from build123d import *

# Parameters (mm, degrees)
SKETCH_1_W          = 101
SKETCH_1_H          = 130
EXTRUDE_1_DEPTH     = 11
CUT_EXTRUDE_1_DEPTH = 8
CUT_EXTRUDE_2_DEPTH = 8
CUT_EXTRUDE_3_REACH = 1271.625
SKETCH_4_W          = 4
SKETCH_4_H          = 32
CUT_EXTRUDE_4_REACH = 1273.161
SKETCH_5_W          = 4
SKETCH_5_H          = 32
SKETCH_6_R          = 36
EXTRUDE_2_DEPTH     = 5
SKETCH_7_R          = 14
EXTRUDE_3_DEPTH     = 4.5
SKETCH_8_R          = 32
CUT_EXTRUDE_5_DEPTH = 5
SKETCH_9_R          = 11
CUT_EXTRUDE_6_DEPTH = 5.6
SKETCH_10_R         = 9
CUT_EXTRUDE_7_DEPTH = 0.5
HOLE_WIZARD_M6_1_D  = 5
FILLET_1_R          = 5
CHAMFER_1_SIZE      = 1
FILLET_2_R          = 2
FILLET_3_R          = 4
FILLET_4_R          = 10


with BuildPart() as part:
    # 草图1 → 凸台-拉伸1 (new body)
    with BuildSketch(Plane(origin=(1263, 0, 0), x_dir=(0, 0, -1), z_dir=(1, 0, 0))):
        with Locations((11, -6.6)):
            Rectangle(SKETCH_1_W, SKETCH_1_H)
    extrude(amount=-EXTRUDE_1_DEPTH)

    # 草图2 → 切除-拉伸1 (cut)
    with BuildSketch(Plane(origin=(1263, 0, 0), x_dir=(0, 0, -1), z_dir=(1, 0, 0))):
        with BuildLine():
            Line((44.5, 25.256406461), (44.5, 42.4))
            Line((44.5, 42.4), (-14.5, 42.4))
            Line((-14.5, 42.4), (-14.5, 15.4))
            Line((-14.5, 15.4), (-34.5, 15.4))
            Line((-34.5, 15.4), (-34.5, -48.6))
            ThreePointArc((-34.5, -48.6), (-29.227922061, -61.327922061), (-16.5, -66.6))
            Line((-16.5, -66.6), (38.5, -66.6))
            ThreePointArc((38.5, -66.6), (51.227922061, -61.327922061), (56.5, -48.6))
            Line((56.5, -48.6), (56.5, 15.458447489))
            ThreePointArc((56.5, 15.458447489), (48.17544468, 17.510439768), (44.5, 25.256406461))
        make_face()
    extrude(amount=-CUT_EXTRUDE_1_DEPTH, mode=Mode.SUBTRACT)

    # 草图3 → 切除-拉伸2 (cut)
    with BuildSketch(Plane(origin=(1263, 0, 0), x_dir=(0, 0, -1), z_dir=(1, 0, 0))):
        with BuildLine():
            Line((42, 55.4), (-20, 55.4))
            ThreePointArc((-20, 55.4), (-25, 50.4), (-20, 45.4))
            Line((-20, 45.4), (42, 45.4))
            ThreePointArc((42, 45.4), (47, 50.4), (42, 55.4))
        make_face()
    extrude(amount=-CUT_EXTRUDE_2_DEPTH, mode=Mode.SUBTRACT)

    # 草图4 → 切除-拉伸3 (cut, up to next)
    with BuildSketch(Plane.XZ.offset(-42.4), mode=Mode.PRIVATE) as cut_extrude_3_sk1:
        with Locations((1261, -11)):
            Rectangle(SKETCH_4_W, SKETCH_4_H)
    cut_extrude_3_tool1 = extrude(cut_extrude_3_sk1.sketch, amount=-CUT_EXTRUDE_3_REACH, mode=Mode.PRIVATE) & part.part
    add(cut_extrude_3_tool1.solids().sort_by_distance((1261, 42.4, -11))[0], mode=Mode.SUBTRACT)

    # 草图5 → 切除-拉伸4 (cut, up to next)
    with BuildSketch(Plane(origin=(0, 58.4, 0), x_dir=(-1, 0, 0), z_dir=(0, 1, 0)), mode=Mode.PRIVATE) as cut_extrude_4_sk1:
        with Locations((-1261, -11)):
            Rectangle(SKETCH_5_W, SKETCH_5_H)
    cut_extrude_4_tool1 = extrude(cut_extrude_4_sk1.sketch, amount=-CUT_EXTRUDE_4_REACH, mode=Mode.PRIVATE) & part.part
    add(cut_extrude_4_tool1.solids().sort_by_distance((1261, 58.4, -11))[0], mode=Mode.SUBTRACT)

    # 草图6 → 凸台-拉伸2 (add)
    with BuildSketch(Plane.ZY.offset(-1252)):
        with Locations((-11, -25.6)):
            Circle(SKETCH_6_R)
    extrude(amount=EXTRUDE_2_DEPTH)

    # 草图7 → 凸台-拉伸3 (add)
    with BuildSketch(Plane.ZY.offset(-1247)):
        with Locations(Location((-11, -25.6, 0), (0, 0, 180))):
            Circle(SKETCH_7_R)
    extrude(amount=EXTRUDE_3_DEPTH)

    # 草图8 → 切除-拉伸5 (cut)
    with BuildSketch(Plane(origin=(1255, 0, 0), x_dir=(0, 0, -1), z_dir=(1, 0, 0))):
        with Locations(Location((11, -25.6, 0), (0, 0, 180))):
            Circle(SKETCH_8_R)
    extrude(amount=-CUT_EXTRUDE_5_DEPTH, mode=Mode.SUBTRACT)

    # 草图9 → 切除-拉伸6 (cut)
    with BuildSketch(Plane(origin=(1250, 0, 0), x_dir=(0, 0, -1), z_dir=(1, 0, 0))):
        with Locations(Location((11, -25.6, 0), (0, 0, 180))):
            Circle(SKETCH_9_R)
    extrude(amount=-CUT_EXTRUDE_6_DEPTH, mode=Mode.SUBTRACT)

    # 草图10 → 切除-拉伸7 (cut)
    with BuildSketch(Plane(origin=(1244.4, 0, 0), x_dir=(0, 0, -1), z_dir=(1, 0, 0))):
        with Locations(Location((11, -25.6, 0), (0, 0, 180))):
            Circle(SKETCH_10_R)
    extrude(amount=-CUT_EXTRUDE_7_DEPTH, mode=Mode.SUBTRACT)

    # M6 螺纹孔1 (through all)
    with Locations(Plane(origin=(1263, 0, 0), x_dir=(0, 0, -1), z_dir=(1, 0, 0))):
        with Locations((53.5, 41.4), (-25.5, 41.4), (-25.5, 21.4), (-33.5, -65.6), (55.5, -65.6), (53.5, 21.4)):
            Hole(HOLE_WIZARD_M6_1_D / 2)

    # 圆角1
    fillet_1_edges = [part.edges().sort_by_distance(p)[0] for p in [
        (1257.5, -71.6, 39.5),
        (1257.5, 58.4, 39.5),
        (1257.5, 58.4, -61.5),
        (1257.5, -71.6, -61.5),
    ]]
    fillet(fillet_1_edges, radius=FILLET_1_R)

    # 倒角1
    chamfer_1_edges = [part.edges().sort_by_distance(p)[0] for p in [
        (1252, -6.6, -61.5),
        (1252, 58.4, -11),
        (1252, -71.6, -11),
        (1252, -6.6, 39.5),
        (1252, -70.135533906, 38.035533906),
        (1252, 56.935533906, 38.035533906),
        (1252, -70.135533906, -60.035533906),
        (1252, 56.935533906, -60.035533906),
        (1255, -25.6, -43),
        (1250, -25.6, -22),
    ]]
    chamfer(chamfer_1_edges, length=CHAMFER_1_SIZE)

    # 圆角2
    fillet_2_edges = [part.edges().sort_by_distance(p)[0] for p in [
        (1252, -25.6, -47),
        (1247, -25.6, -47),
        (1247, -25.6, 3),
        (1242.5, -25.6, 3),
    ]]
    fillet(fillet_2_edges, radius=FILLET_2_R)

    # 圆角3
    fillet_3_edges = [part.edges().sort_by_distance(p)[0] for p in [
        (1259, 15.458447489, -56.5),
        (1259, 15.4, 34.5),
        (1259, 42.4, 14.5),
        (1259, 42.4, -44.5),
    ]]
    fillet(fillet_3_edges, radius=FILLET_3_R)

    # 圆角4
    fillet_4_edges = [part.edges().sort_by_distance(p)[0] for p in [
        (1259, 15.4, 14.5),
    ]]
    fillet(fillet_4_edges, radius=FILLET_4_R)


solid = part.part
Verification items for the finished model (mm, model axes). A direction names the side the tool comes from. Coordinates: 2 decimals unless noted, no trailing zeros. Order: outer loops, then holes, each group sorted by start corner. A loop starts at its lowest first (then second) coordinate and runs counter-clockwise, first axis right, second up. Notation, with made-up numbers: M 36,61.25 L 56,61.25 A18 ccw 56,89.25 Z; hole C 21,-9 d3. An arc over 180 degrees is marked long. Return JSON: item names as keys, results as strings.
1) Gauge pin test, flat ends, axial feed: pin 1 (1.5 mm diameter, centred on y = 26, z = 19.5, fed in from -X); pin 2 (4 mm diameter, centred on x = 1249, y = 14.5, fed in from +Z); pin 3 (12 mm diameter, centred on x = 1252, y = -1, fed in from +Z); pin 4 (1 mm diameter, centred on x = 1248.5, z = -8.5, fed in from +Y). Record the tip position at first contact, or that the pin passes through.
Answer list:
{"pin 1": "x = 1252", "pin 2": "through", "pin 3": "z = 39.5", "pin 4": "y = 10.33"}
2) Cross-section at A-A, the plane z = 32.5. Record the boundary of the cut face in (x, y), and give its area (3 significant figures).
Answer list:
{"outline": "M 1252,-70.6 L 1253,-71.6 L 1263,-71.6 L 1263,-67.89 L 1252,-67.89 Z; M 1252,-63.31 L 1263,-63.31 L 1263,-56.85 L 1255,-56.85 L 1255,14.86 L 1263,14.86 L 1263,58.4 L 1253,58.4 L 1252,57.4 Z", "area": "805 mm2"}
3) Access from +Z, -Z, +X, -X, +Y, -Y to the whole of each face (thin tool, end or side, straight path). Record for faces 1 (the flat face through (1261, 57, 5)), 2 (the cylindrical face through (1244.75, -11.93, -7.97)), 3 (the cylindrical face through (1259.1, 50.3, -47)).
Answer list:
{"face 1": "+X, +Y", "face 2": "-X", "face 3": "+X"}
4) Cross-section at B-B, the plane y = 21.4. Record the boundary of the cut face in (x, z).
Answer list:
{"outline": "M 1252,-60.5 L 1253,-61.5 L 1263,-61.5 L 1263,-56 L 1252,-56 Z; M 1252,-51 L 1263,-51 L 1263,-45.27 L 1255,-45.27 L 1255,15.33 L 1263,15.33 L 1263,23 L 1252,23 Z; M 1252,28 L 1263,28 L 1263,39.5 L 1253,39.5 L 1252,38.5 Z"}
5) Cross-section at C-C, the plane y = 35. Record the boundary of the cut face in (x, z).
Answer list:
{"outline": "M 1252,-60.5 L 1253,-61.5 L 1263,-61.5 L 1263,-44.5 L 1255,-44.5 L 1255,14.5 L 1263,14.5 L 1263,39.5 L 1253,39.5 L 1252,38.5 Z"}
6) Thickness scan on L1, parallel to Y at x = 1254.75, z = 25.5; L2, parallel to Y at x = 1256.25, z = -23.5; L3, parallel to Z at x = 1256.75, y = -8. Record the ranges inside material, lowest first. Write a range as [from, to].
Answer list:
{"L1": "[-71.6, 18.9], [23.9, 38.9], [43.9, 58.4]", "L2": "[-71.6, -66.6], [42.4, 45.4], [55.4, 58.4]", "L3": "[-61.5, -56.5], [34.5, 39.5]"}
